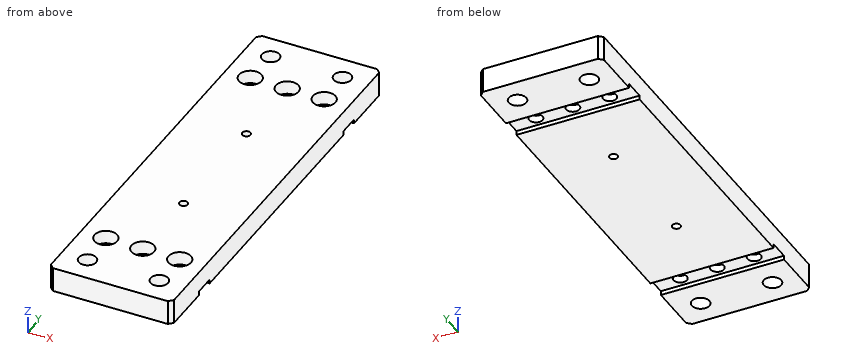
from build123d import *

# Parameters (mm, degrees)
SKETCH1_W                                            = 60
SKETCH1_H                                            = 200
BOSS_EXTRUDE1_DEPTH                                  = 6
CHAMFER1_SIZE                                        = 2
SKETCH2_W                                            = 60
SKETCH2_H                                            = 10
CUT_EXTRUDE1_DEPTH                                   = 2
HOLE_SIZE_PER_SOCKET_HEAD_CAP_SCREW_TYPE_D           = 6.5
HOLE_SIZE_PER_SOCKET_HEAD_CAP_SCREW_TYPE_CBORE_D     = 11
HOLE_SIZE_PER_SOCKET_HEAD_CAP_SCREW_TYPE_CBORE_DEPTH = 6.5
SKETCH5_R                                            = 4.25
CUT_EXTRUDE2_DEPTH                                   = 106.090437243
SKETCH6_R                                            = 2
CUT_EXTRUDE3_DEPTH                                   = 106.090437243


with BuildPart() as part:
    # Sketch1 → Boss-Extrude1 (new, symmetric)
    with BuildSketch(Plane.XY):
        Rectangle(SKETCH1_W, SKETCH1_H)
    extrude(amount=BOSS_EXTRUDE1_DEPTH, both=True)

    # Chamfer1
    chamfer1_edges = [part.edges().sort_by_distance(p)[0] for p in [
        (30, -100, 0),
        (-30, -100, 0),
        (-30, 100, 0),
        (30, 100, 0),
    ]]
    chamfer(chamfer1_edges, length=CHAMFER1_SIZE)

    # Sketch2 → Cut-Extrude1 (cut)
    with BuildSketch(Plane(origin=(0, 0, -6), x_dir=(-1, 0, 0), z_dir=(0, 0, -1))):
        with Locations((0, 69)):
            Rectangle(SKETCH2_W, SKETCH2_H)
        with Locations((0, -69)):
            Rectangle(SKETCH2_W, SKETCH2_H)
    extrude(amount=-CUT_EXTRUDE1_DEPTH, mode=Mode.SUBTRACT)

    # Hole size per socket head cap screw type 1 (through all)
    with Locations(Plane.XY.offset(6)):
        with Locations((-18, -69), (0, -69), (18, -69), (18, 69), (0, 69), (-18, 69)):
            CounterBoreHole(HOLE_SIZE_PER_SOCKET_HEAD_CAP_SCREW_TYPE_D / 2, HOLE_SIZE_PER_SOCKET_HEAD_CAP_SCREW_TYPE_CBORE_D / 2, HOLE_SIZE_PER_SOCKET_HEAD_CAP_SCREW_TYPE_CBORE_DEPTH)

    # Sketch5 → Cut-Extrude2 (cut, through all)
    with BuildSketch(Plane(origin=(0, 0, -6), x_dir=(-1, 0, 0), z_dir=(0, 0, -1))):
        with Locations((17.5, 87.5)):
            Circle(SKETCH5_R)
        with Locations((-17.5, 87.5)):
            Circle(SKETCH5_R)
        with Locations((17.5, -87.5)):
            Circle(SKETCH5_R)
        with Locations((-17.5, -87.5)):
            Circle(SKETCH5_R)
    extrude(amount=-CUT_EXTRUDE2_DEPTH, mode=Mode.SUBTRACT)

    # Sketch6 → Cut-Extrude3 (cut, through all)
    with BuildSketch(Plane.XY.offset(6)):
        with Locations((0, 30)):
            Circle(SKETCH6_R)
        with Locations((0, -30)):
            Circle(SKETCH6_R)
    extrude(amount=-CUT_EXTRUDE3_DEPTH, mode=Mode.SUBTRACT)


solid = part.part
The listing builds one solid part. Answer for the finished solid, in the listing's coordinates (mm). Round coordinates to 2 decimals unless told otherwise and drop trailing zeros. Write each loop counter-clockwise with the first axis right and the second up, starting at its lowest first coordinate (ties: lowest second). Pieces come first, ordered by that corner, then holes. Notation, with made-up numbers: (-36, 62.25) - (23, 62.25) arc R27 cw to (23, 81.25) - close; hole circle Ø11 at (53, 29.5). An arc over 180 degrees is marked (long way). Use a Markdown table: item, result. Add a question column.
1. Consider line 1 (Y direction, x = -18, z = 3.25); line 2 (Y direction, x = -6, z = -4.25); line 3 (Y direction, x = -18, z = -1.4). Determine where each line is inside the solid, lowest interval first.
2. Flat-ended cylindrical pins translate along their axes: P1, Ø3.5, axis at x = -2.5, y = -66.5, coming from the +Z side; P2, Ø9, axis at x = 18, y = -69, coming from the -Z side; P3, Ø7, axis at x = 17.5, y = -87.5, coming from the +Z side. Find the tip coordinate at first contact, or state that the pin passes through.
3. The part is cut by section C-C (y = -87.5). Write down the section's boundary in (x, z), and give its area (3 significant figures).
4. The part is cut by section B-B (y = 30). Write down the section's boundary in (x, z).
5. The part is cut by section D-D (x = 8). Write down the section's boundary in (y, z).
6. The part is cut by section A-A (y = 69). Write down the section's boundary in (x, z), and give its area (3 significant figures).
Reported:
| question | item | result |
|---|---|---|
| 1 | line 1 | -100 to -91.72, -83.28 to -74.5, -63.5 to 63.5, 74.5 to 83.28, 91.72 to 100 |
| 1 | line 2 | -100 to -74, -64 to 64, 74 to 100 |
| 1 | line 3 | -100 to -91.72, -83.28 to -72.25, -65.75 to 65.75, 72.25 to 83.28, 91.72 to 100 |
| 2 | P1 | z = -0.5 |
| 2 | P2 | z = -4 |
| 2 | P3 | through |
| 3 | outline | (-30, -6) - (-21.75, -6) - (-21.75, 6) - (-30, 6) - close; (-13.25, -6) - (13.25, -6) - (13.25, 6) - (-13.25, 6) - close; (21.75, -6) - (30, -6) - (30, 6) - (21.75, 6) - close |
| 3 | area | 516 mm^2 |
| 4 | outline | (-30, -6) - (-2, -6) - (-2, 6) - (-30, 6) - close; (2, -6) - (30, -6) - (30, 6) - (2, 6) - close |
| 5 | outline | (-100, -6) - (-74, -6) - (-74, -4) - (-64, -4) - (-64, -6) - (64, -6) - (64, -4) - (74, -4) - (74, -6) - (100, -6) - (100, 6) - (-100, 6) - close |
| 6 | outline | (-30, -4) - (-21.25, -4) - (-21.25, -0.5) - (-23.5, -0.5) - (-23.5, 6) - (-30, 6) - close; (-14.75, -4) - (-3.25, -4) - (-3.25, -0.5) - (-5.5, -0.5) - (-5.5, 6) - (-12.5, 6) - (-12.5, -0.5) - (-14.75, -0.5) - close; (3.25, -4) - (14.75, -4) - (14.75, -0.5) - (12.5, -0.5) - (12.5, 6) - (5.5, 6) - (5.5, -0.5) - (3.25, -0.5) - close; (21.25, -4) - (30, -4) - (30, 6) - (23.5, 6) - (23.5, -0.5) - (21.25, -0.5) - close |
| 6 | area | 317 mm^2 |
